Build history of the part. All positions in model axes, mm. Face numbers are marked on the shaded views. A direction names the side the tool comes from. Round coordinates to 2 decimals unless told otherwise and drop trailing zeros. Write each loop counter-clockwise with the first axis right and the second up, starting at its lowest first coordinate (ties: lowest second). Pieces come first, ordered by that corner, then holes. Notation, with made-up numbers: (-24, 80.5) -> (-8, 80.5) arc R23 cw to (-8, 119.5) -> close; hole circle Ø6 at (1.5, -33.5). An arc over 180 degrees is marked (long way). Answer in a Markdown table with one row per item. Add a question column.
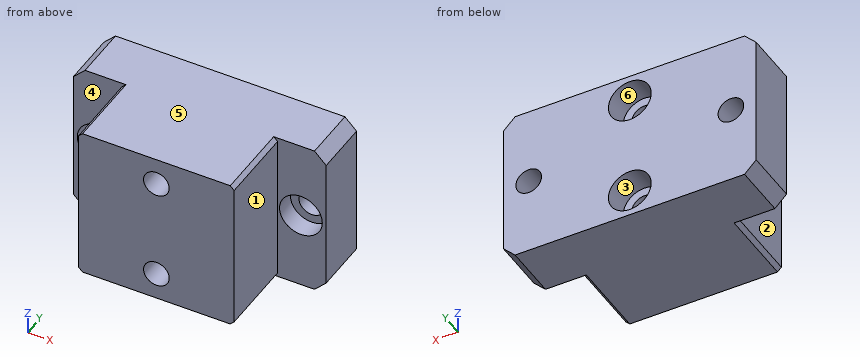
from build123d import *

# Parameters (mm, degrees)
SKETCH_1_W                  = 65
SKETCH_1_H                  = 40
EXTRUDE_1_DEPTH             = 17
HOLE_WIZARD_2_D             = 6.6
HOLE_WIZARD_2_CBORE_D       = 11
HOLE_WIZARD_2_CBORE_DEPTH   = 6.8
CHAMFER_1_SIZE              = 3
SKETCH_6_OUTSIDE_W          = 83.71
SKETCH_6_OUTSIDE_H          = 58.71
SKETCH_6_OUTSIDE_W_2        = 40
SKETCH_6_OUTSIDE_H_2        = 40
CUT_EXTRUDE_1_DEPTH         = 20
HOLE_WIZARD_2_2_D           = 6.6
HOLE_WIZARD_2_2_CBORE_D     = 11
HOLE_WIZARD_2_2_CBORE_DEPTH = 5
CHAMFER_2_SIZE              = 1


with BuildPart() as part:
    # 草图1 → 凸台-拉伸1 (new, symmetric)
    with BuildSketch(Plane(origin=(0, 0, 0), x_dir=(1, 0, 0), z_dir=(0, 1, 0))):
        Rectangle(SKETCH_1_W, SKETCH_1_H)
    extrude(amount=EXTRUDE_1_DEPTH, both=True)

    # Hole Wizard 2 (through all)
    with Locations(Plane(origin=(0, 17, 0), x_dir=(1, 0, 0), z_dir=(0, 1, 0))):
        with Locations((0, -13), (0, 13)):
            CounterBoreHole(HOLE_WIZARD_2_D / 2, HOLE_WIZARD_2_CBORE_D / 2, HOLE_WIZARD_2_CBORE_DEPTH)

    # 倒角1
    chamfer_1_edges = [part.edges().sort_by_distance(p)[0] for p in [
        (32.5, 0, 20),
        (-32.5, 0, 20),
        (-32.5, 0, -20),
        (32.5, 0, -20),
    ]]
    chamfer(chamfer_1_edges, length=CHAMFER_1_SIZE)

    # 草图6 outside → 切除-拉伸1 (cut)
    with BuildSketch(Plane.XZ.offset(17)):
        Rectangle(SKETCH_6_OUTSIDE_W, SKETCH_6_OUTSIDE_H)
        Rectangle(SKETCH_6_OUTSIDE_W_2, SKETCH_6_OUTSIDE_H_2, mode=Mode.SUBTRACT)
    extrude(amount=-CUT_EXTRUDE_1_DEPTH, mode=Mode.SUBTRACT)

    # Hole Wizard 2 2 (through all)
    with Locations(Plane.XZ.offset(-3)):
        with Locations((26, 0), (-26, 0)):
            CounterBoreHole(HOLE_WIZARD_2_2_D / 2, HOLE_WIZARD_2_2_CBORE_D / 2, HOLE_WIZARD_2_2_CBORE_DEPTH)

    # 倒角2
    chamfer_2_edges = [part.edges().sort_by_distance(p)[0] for p in [
        (-20, -7, 20),
        (20, -7, 20),
        (20, -7, -20),
        (-20, -7, -20),
    ]]
    chamfer(chamfer_2_edges, length=CHAMFER_2_SIZE)


solid = part.part
(1) Drop flat-ended pins along their axis: P1, Ø7, axis at x = -25, z = -5, coming from the -Y side; P2, Ø8.5, axis at x = 26, z = 0, coming from the -Y side; P3, Ø10.5, axis at x = 0, z = -13, coming from the +Y side. Give the stop position or say it passes through.
(2) Saw through at D-D (x = 0). List the corners of the cut face in (y, z).
(3) Saw through at B-B (z = 13). List the corners of the cut face in (x, y), plus the area to 3 significant figures.
(4) Which spindle directions (+Z, -Z, +X, -X, +Y, -Y) get a long thin tool onto all of the face, cutting with end or side? Do the marked faces 1, 2 and 3. Say none if no direction does.
(5) Mould opens along Z. For the marked faces 4, 5 and 6 say: pulls with the +Z half, pulls with the -Z half, needs draft (parallel to the pull), parting line crosses it, or undercut.
(6) Probe line 1 along Z through (x, y) = (0, 15); line 2 along Z through (x, y) = (0, -0.25); line 3 along Z through (x, y) = (-26, 13). List the from-to ranges inside material, lowest first.
(7) Saw through at A-A (x = 26). List the corners of the cut face in (y, z).
(8) Saw through at C-C (y = 13). List the corners of the cut face in (x, z), plus the area to 3 significant figures.
Answer sheet:
| question | item | result |
|---|---|---|
| 1 | P1 | stops at y = 3 |
| 1 | P2 | stops at y = 8 |
| 1 | P3 | stops at y = 10.2 |
| 2 | outline | (-17, -20) -> (17, -20) -> (17, -18.5) -> (10.2, -18.5) -> (10.2, -16.3) -> (-17, -16.3) -> close; (-17, -9.7) -> (10.2, -9.7) -> (10.2, -7.5) -> (17, -7.5) -> (17, 7.5) -> (10.2, 7.5) -> (10.2, 9.7) -> (-17, 9.7) -> close; (-17, 16.3) -> (10.2, 16.3) -> (10.2, 18.5) -> (17, 18.5) -> (17, 20) -> (-17, 20) -> close |
| 3 | outline | (-32.5, 3) -> (-20, 3) -> (-20, -17) -> (-3.3, -17) -> (-3.3, 10.2) -> (-5.5, 10.2) -> (-5.5, 17) -> (-32.5, 17) -> close; (3.3, -17) -> (20, -17) -> (20, 3) -> (32.5, 3) -> (32.5, 17) -> (5.5, 17) -> (5.5, 10.2) -> (3.3, 10.2) -> close |
| 3 | area | 1,460 mm² |
| 4 | face 1 | +Z, -Z, +X, -Y |
| 4 | face 2 | +Z, -Z, -X, -Y |
| 4 | face 3 | +Y |
| 5 | face 4 | needs draft |
| 5 | face 5 | pulls with the +Z half |
| 5 | face 6 | undercut |
| 6 | line 1 | z = -20 to -18.5, -7.5 to 7.5, 18.5 to 20 |
| 6 | line 2 | z = -20 to -16.3, -9.7 to 9.7, 16.3 to 20 |
| 6 | line 3 | z = -20 to -3.3, 3.3 to 20 |
| 7 | outline | (3, -20) -> (17, -20) -> (17, -3.3) -> (8, -3.3) -> (8, -5.5) -> (3, -5.5) -> close; (3, 5.5) -> (8, 5.5) -> (8, 3.3) -> (17, 3.3) -> (17, 20) -> (3, 20) -> close |
| 8 | outline | (-32.5, -17) -> (-29.5, -20) -> (29.5, -20) -> (32.5, -17) -> (32.5, 17) -> (29.5, 20) -> (-29.5, 20) -> (-32.5, 17) -> close; hole circle Ø6.6 at (-26, 0); hole circle Ø11 at (0, -13); hole circle Ø11 at (0, 13); hole circle Ø6.6 at (26, 0) |
| 8 | area | 2,320 mm² |
